For this review, use the dimensioned drawing (mm, ordinates from the lowest corner) and the shaded views. Give positions to 0.01 mm unless a question says otherwise; leave off trailing zeros. Order: outer loops, then holes, each group sorted by start corner. A loop starts at its lowest first (then second) coordinate and runs counter-clockwise, first axis right, second up.
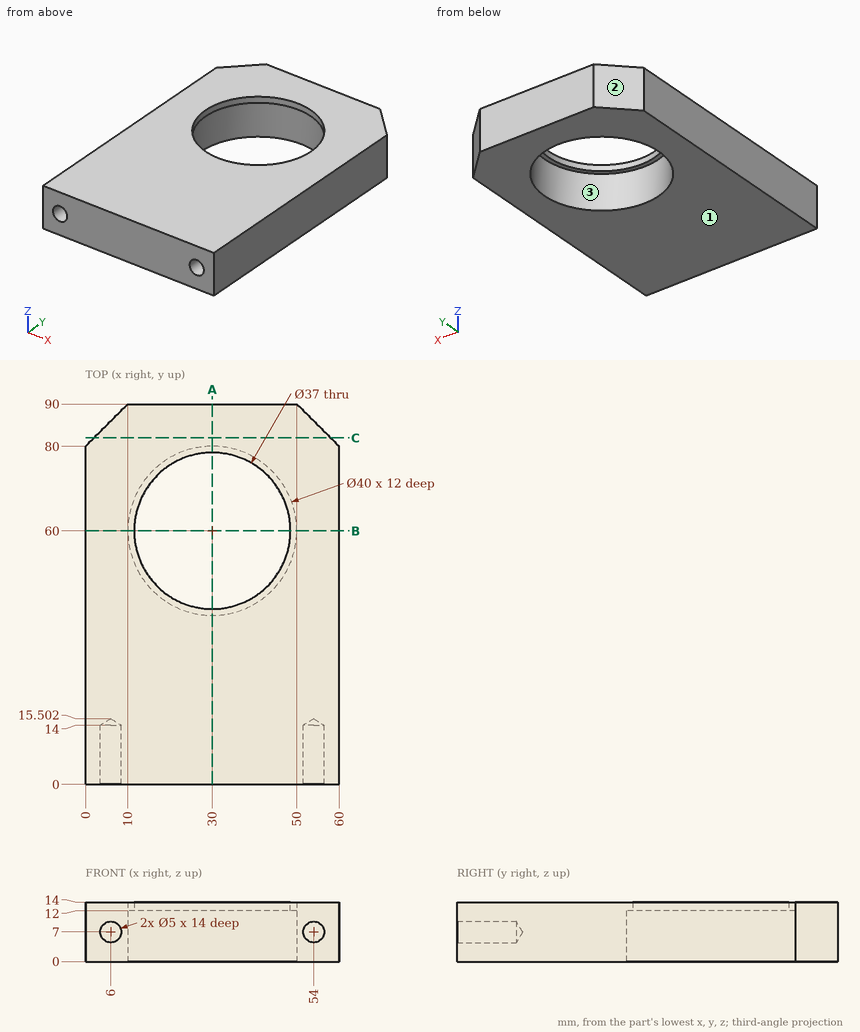
1. Draft analysis for pull direction X (two halves, no side actions). For the marked faces 1, 2 and 3, state which applies: pulls with the +X half, pulls with the -X half, needs draft (parallel to the pull), parting line crosses it, or undercut.
2. To check wall thickness, follow line 1 (Y direction, x = 30, z = 5.25); line 2 (X direction, y = 9, z = 7); line 3 (X direction, y = 53, z = 0.5) (1 decimal). State the ranges of each line that lie inside material, in increasing order.
3. Take a section at B-B (y = 60). Write out the cut boundary in (x, z).
4. Take a section at C-C (y = 82). Write out the cut boundary in (x, z).
5. Insertion check: pin 1 (4 mm diameter, centred on x = 54, z = 7, fed in from +Y); pin 2 (3 mm diameter, centred on x = 6, z = 7, fed in from -Y). Each pin has a flat end and moves straight along its axis. Give the tip position at first contact, or say it passes through.
6. Take a section at A-A (x = 30). Write out the cut boundary in (y, z), and give its area (3 significant figures).
Answer:
1. face 1: needs draft
1. face 2: pulls with the -X half
1. face 3: undercut
2. line 1: y = 0 to 40, 80 to 90
2. line 2: x = 0 to 3.5, 8.5 to 51.5, 56.5 to 60
2. line 3: x = 0 to 11.3, 48.7 to 60
3. outline: (0, 0) - (10, 0) - (10, 12) - (11.5, 12) - (11.5, 14) - (0, 14) - close; (48.5, 12) - (50, 12) - (50, 0) - (60, 0) - (60, 14) - (48.5, 14) - close
4. outline: (2, 0) - (58, 0) - (58, 14) - (2, 14) - close
5. pin 1: stops at y = 88
5. pin 2: stops at y = 14.6
6. outline: (0, 0) - (40, 0) - (40, 12) - (41.5, 12) - (41.5, 14) - (0, 14) - close; (78.5, 12) - (80, 12) - (80, 0) - (90, 0) - (90, 14) - (78.5, 14) - close
6. area: 706 mm2
